Job drawing, mm, ordinate dimensions from the low corner. One solid piece. Give positions to 0.01 mm unless a question says otherwise; leave off trailing zeros. Order: outer loops, then holes, each group sorted by start corner. A loop starts at its lowest first (then second) coordinate and runs counter-clockwise, first axis right, second up. Notation, with made-up numbers: (46.5, 36.25) -> (65.5, 36.25) arc R18 cw to (65.5, 63.25) -> close; hole circle Ø4 at (-38.5, 77). An arc over 180 degrees is marked (long way). Write item = value, one per line. Start each with the question number.
(1) Saw through at B-B, the plane y = 80. List the corners of the cut face in (x, z), then the cut area to 3 significant figures.
(2) Saw through at C-C, the plane z = 3.75. List the corners of the cut face in (x, y) (1 decimal), then the cut area to 3 significant figures.
(3) Probe line 1 along Y through (x, z) = (120, 2.5); line 2 along Z through (x, y) = (69.5, 442.5); line 3 along Y through (x, z) = (115, 3.5) (1 decimal). List the from-to ranges inside material, lowest first. Write a range as from..to.
(4) Saw through at A-A, the plane x = 120. List the corners of the cut face in (y, z), then the cut area to 3 significant figures.
(5) Flat gauge pins, fed straight in: pin 1 (8 mm diameter, centred on x = 182, y = 172.5, fed in from +Z); pin 2 (9 mm diameter, centred on x = 37, z = 4, fed in from +Y); pin 3 (1.5 mm diameter, centred on x = 91, z = 2.5, fed in from +Y) (1 decimal). Where does each tip first touch, or does it go through?
(6) Two-plate mould, pull along Z, no slides. Class the marked faces 1 and 2: pulls with the +Z half, pulls with the -Z half, needs draft (parallel to the pull), parting line crosses it, or undercut.
(7) Saw through at D-D, the plane x = 205. List the corners of the cut face in (y, z), then the cut area to 3 significant figures.
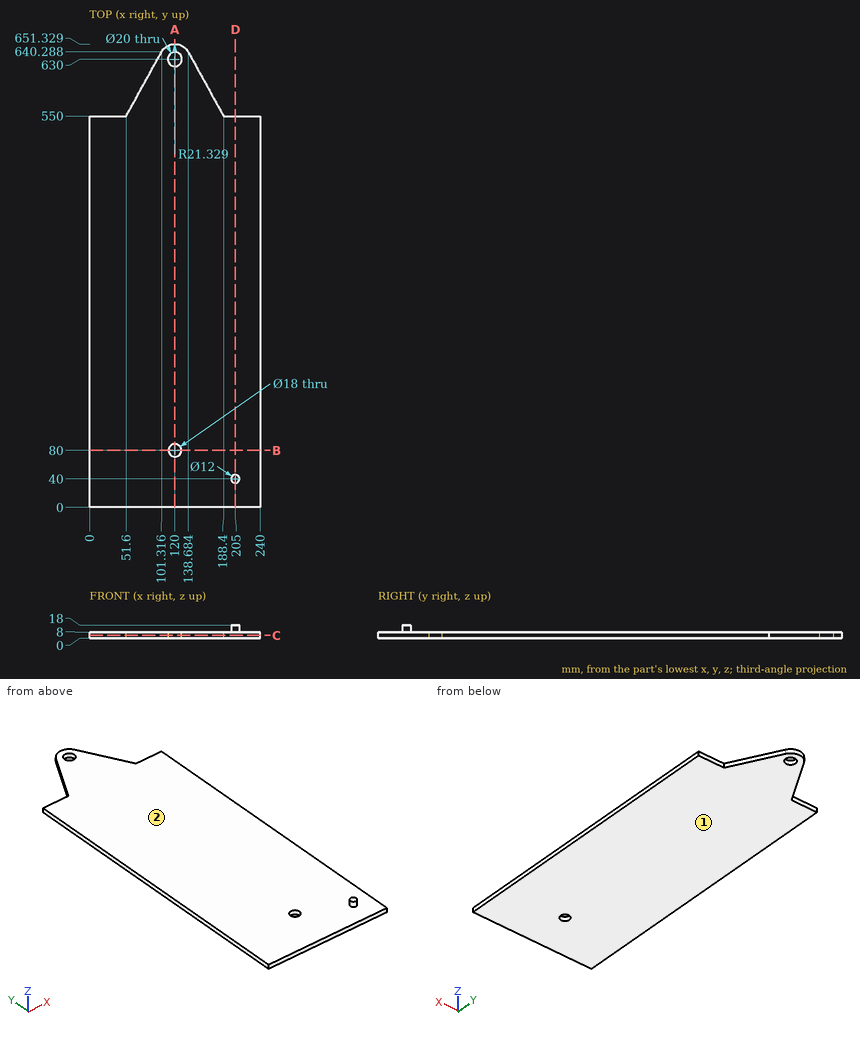
Results list:
q1.outline = (0, 0) -> (111, 0) -> (111, 8) -> (0, 8) -> close; (129, 0) -> (240, 0) -> (240, 8) -> (129, 8) -> close
q1.area = 1,780 mm^2
q2.outline = (0, 0) -> (240, 0) -> (240, 550) -> (188.4, 550) -> (138.7, 640.3) arc R21.3 ccw to (101.3, 640.3) -> (51.6, 550) -> (0, 550) -> close; hole circle Ø20 at (120, 630); hole circle Ø18 at (120, 80)
q2.area = 140,000 mm^2
q3.line_1 = 0..71, 89..620, 640..651.33
q3.line_2 = 0..8
q3.line_3 = 0..72.5, 87.5..621.3, 638.7..650.7
q4.outline = (0, 0) -> (71, 0) -> (71, 8) -> (0, 8) -> close; (89, 0) -> (620, 0) -> (620, 8) -> (89, 8) -> close; (640, 0) -> (651.33, 0) -> (651.33, 8) -> (640, 8) -> close
q4.area = 4,910 mm^2
q5.pin_1 = 8
q5.pin_2 = 550
q5.pin_3 = 622.9
q6.face_1 = pulls with the -Z half
q6.face_2 = pulls with the +Z half
q7.outline = (0, 0) -> (550, 0) -> (550, 8) -> (46, 8) -> (46, 18) -> (34, 18) -> (34, 8) -> (0, 8) -> close
q7.area = 4,520 mm^2
